Verification items for the finished model (mm, model axes). A direction names the side the tool comes from. Coordinates: 2 decimals unless noted, no trailing zeros. Write each loop counter-clockwise with the first axis right and the second up, starting at its lowest first coordinate (ties: lowest second). Pieces come first, ordered by that corner, then holes. Notation, with made-up numbers: M -25,57.25 L 5,57.25 A22 cw 5,87.25 Z; hole C -28.75,-25.5 d4. An arc over 180 degrees is marked long. Answer in a Markdown table with one row per item.
from build123d import *

# Parameters (mm, degrees)
SKETCH1_W           = 550
SKETCH1_H           = 50
BOSS_EXTRUDE1_DEPTH = 10
SKETCH2_R           = 17.5
CUT_EXTRUDE1_DEPTH  = 10
CUT_EXTRUDE2_DEPTH  = 10
FILLET1_R           = 20


with BuildPart() as part:
    # Sketch1 → Boss-Extrude1 (new body)
    with BuildSketch(Plane.XY):
        Rectangle(SKETCH1_W, SKETCH1_H)
    extrude(amount=BOSS_EXTRUDE1_DEPTH)

    # Sketch2 → Cut-Extrude1 (cut)
    with BuildSketch(Plane.XY.offset(10)):
        with Locations((-250, 0)):
            Circle(SKETCH2_R)
    extrude(amount=-CUT_EXTRUDE1_DEPTH, mode=Mode.SUBTRACT)

    # Sketch3 → Cut-Extrude2 (cut)
    with BuildSketch(Plane.XY.offset(10)):
        with BuildLine():
            Line((250.099813904, -5.340973555), (134.099813904, -5.340973555))
            ThreePointArc((134.099813904, -5.340973555), (130.917833389, -4.02295407), (129.599813904, -0.840973555))
            Line((129.599813904, -0.840973555), (129.599813904, 0.159026445))
            ThreePointArc((129.599813904, 0.159026445), (130.917833389, 3.341006961), (134.099813904, 4.659026445))
            Line((134.099813904, 4.659026445), (250.099813904, 4.659026445))
            ThreePointArc((250.099813904, 4.659026445), (253.281794419, 3.341006961), (254.599813904, 0.159026445))
            Line((254.599813904, 0.159026445), (254.599813904, -0.840973555))
            ThreePointArc((254.599813904, -0.840973555), (253.281794419, -4.02295407), (250.099813904, -5.340973555))
        make_face()
    extrude(amount=-CUT_EXTRUDE2_DEPTH, mode=Mode.SUBTRACT)

    # Fillet1
    fillet1_edges = [part.edges().sort_by_distance(p)[0] for p in [
        (-275, 25, 5),
        (-275, -25, 5),
    ]]
    fillet(fillet1_edges, radius=FILLET1_R)


solid = part.part
1) Tool access check on faces 1 (the face through (-269.297, 18.986, 5.07)), 2 (the face through (193, -5.341, 5)). Record the directions out of +Z, -Z, +X, -X, +Y, -Y that give a thin tool (end or side, any length) a straight path to the whole face; none if there is none.
Response values:
| item | result |
|---|---|
| face 1 | +Z, -Z, -X, +Y |
| face 2 | +Z, -Z |
2) Thickness scan on L1, parallel to X at y = -1, z = 2.25; L2, parallel to Y at x = -250, z = 5.25; L3, parallel to X at y = -2, z = 6. Record the ranges inside material, lowest first. Write a range as [from, to].
Response values:
| item | result |
|---|---|
| L1 | x = [-275, -267.47], [-232.53, 129.6], [254.6, 275] |
| L2 | y = [-25, -17.5], [17.5, 25] |
| L3 | x = [-275, -267.39], [-232.61, 129.75], [254.45, 275] |
3) Sectioned sample at B-B (z = 4). Record the cut outline in (x, y), then the cut area to 3 significant figures.
Response values:
| item | result |
|---|---|
| outline | M -275,-5 A20 ccw -255,-25 L 275,-25 L 275,25 L -255,25 A20 ccw -275,5 Z; hole C -250,0 d35; hole M 129.6,-0.84 A4.5 ccw 134.1,-5.34 L 250.1,-5.34 A4.5 ccw 254.6,-0.84 L 254.6,0.16 A4.5 ccw 250.1,4.66 L 134.1,4.66 A4.5 ccw 129.6,0.16 Z |
| area | 25,100 mm² |
4) Sectioned sample at A-A (x = -250). Record the cut outline in (y, z), then the cut area to 3 significant figures.
Response values:
| item | result |
|---|---|
| outline | M -25,0 L -17.5,0 L -17.5,10 L -25,10 Z; M 17.5,0 L 25,0 L 25,10 L 17.5,10 Z |
| area | 150 mm² |
5) Release check for a two-part mould opening along Y. For faces 3 (the face through (-4, 0, 0)), 4 (the face through (6, 25, 5)), 5 (the face through (191, 4.659, 5)) record: +Y half, -Y half, draft (parallel to the pull), parting line (faces both ways), or undercut.
Response values:
| item | result |
|---|---|
| face 3 | draft |
| face 4 | +Y half |
| face 5 | undercut |
6) Sectioned sample at C-C (x = 237). Record the cut outline in (y, z), then the cut area to 3 significant figures.
Response values:
| item | result |
|---|---|
| outline | M -25,0 L -5.34,0 L -5.34,10 L -25,10 Z; M 4.66,0 L 25,0 L 25,10 L 4.66,10 Z |
| area | 400 mm² |
